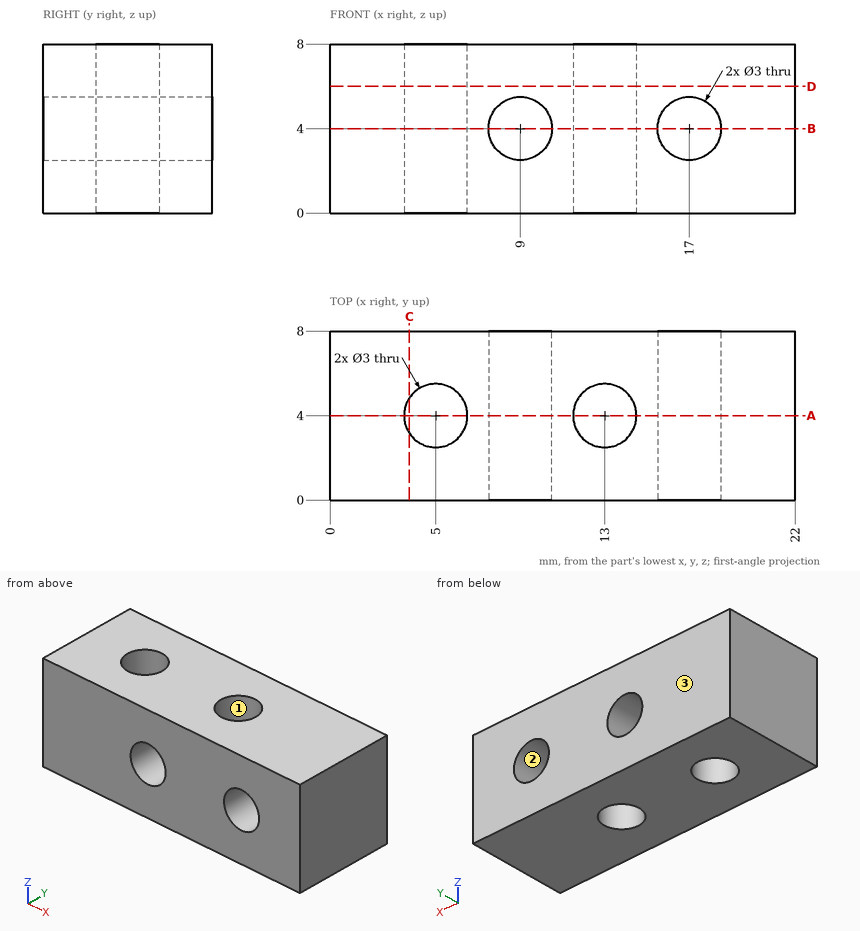
Print and shaded views of the part. All mm, measured from the part's lowest x, y and z. Coordinates: 2 decimals unless noted, no trailing zeros. Order: outer loops, then holes, each group sorted by start corner. A loop starts at its lowest first (then second) coordinate and runs counter-clockwise, first axis right, second up. Notation, with made-up numbers: (36, -13) -> (42, -13) arc R21 ccw to (42, 14) -> close; hole circle Ø5 at (-37.5, 28.5). An arc over 180 degrees is marked (long way). Use one line per item in the form item = value. Start each with the question number.
1) Band-saw the part on A-A on y = 4. Give the cut face in (x, z), then the cut area to 3 significant figures.
2) Pull direction Y, two halves, no side cores. Call the marked faces 1, 2 and 3: +Y half, -Y half, draft (parallel to the pull), parting line (faces both ways), or undercut.
3) Band-saw the part on B-B on z = 4. Give the cut face in (x, y).
4) Drill centre lines: L1, parallel to Y at x = 13, z = 5.25; L2, parallel to X at y = 6, z = 3.75; L3, parallel to X at y = 3.5, z = 1.75. Where is each one in solid material? Low to high. Write a range as [from, to].
5) Band-saw the part on D-D on z = 6. Give the cut face in (x, y).
6) Band-saw the part on C-C on x = 3.75. Give the cut face in (y, z).
7) Drop a flat-ended pin along its axis: pin 1 (2.5 mm diameter, centred on x = 13, y = 4, fed in from -Z). Give the stop position or say it passes through.
Entries:
q1.outline = (0, 0) -> (3.5, 0) -> (3.5, 8) -> (0, 8) -> close; (6.5, 0) -> (11.5, 0) -> (11.5, 8) -> (6.5, 8) -> close; (14.5, 0) -> (22, 0) -> (22, 8) -> (14.5, 8) -> close; hole circle Ø3 at (9, 4); hole circle Ø3 at (17, 4)
q1.area = 114 mm2
q2.face_1 = undercut
q2.face_2 = draft
q2.face_3 = +Y half
q3.outline = (0, 0) -> (7.5, 0) -> (7.5, 8) -> (0, 8) -> close; (10.5, 0) -> (15.5, 0) -> (15.5, 8) -> (10.5, 8) -> close; (18.5, 0) -> (22, 0) -> (22, 8) -> (18.5, 8) -> close; hole circle Ø3 at (5, 4); hole circle Ø3 at (13, 4)
q4.L1 = [0, 2.5], [5.5, 8]
q4.L2 = [0, 7.52], [10.48, 15.52], [18.48, 22]
q4.L3 = [0, 3.59], [6.41, 11.59], [14.41, 22]
q5.outline = (0, 0) -> (22, 0) -> (22, 8) -> (0, 8) -> close; hole circle Ø3 at (5, 4); hole circle Ø3 at (13, 4)
q6.outline = (0, 0) -> (3.17, 0) -> (3.17, 8) -> (0, 8) -> close; (4.83, 0) -> (8, 0) -> (8, 8) -> (4.83, 8) -> close
q7.pin_1 = through
